Input: part model. Units: mm. Frame: model coordinates. A direction names the side the tool comes from. Round coordinates to 2 decimals unless told otherwise and drop trailing zeros. Write each loop counter-clockwise with the first axis right and the second up, starting at its lowest first coordinate (ties: lowest second). Pieces come first, ordered by that corner, then holes. Notation, with made-up numbers: (3, -21.5) -> (19, -21.5) arc R14 ccw to (19, -6.5) -> close; hole circle Ø7 at (28, -38). An arc over 180 degrees is marked (long way). Write item = value, one per line.
```python
from build123d import *

# Parameters (mm, degrees)
SKETCH_1_W      = 35
SKETCH_1_H      = 100
EXTRUDE_1_DEPTH = 10
SKETCH_2_R      = 12.5
EXTRUDE_2_DEPTH = 30
SKETCH_3_R      = 7.5
EXTRUDE_3_DEPTH = 25


with BuildPart() as part:
    # 草图1 → 凸台-拉伸1 (new body)
    with BuildSketch(Plane.XY):
        Rectangle(SKETCH_1_W, SKETCH_1_H)
    extrude(amount=EXTRUDE_1_DEPTH)

    # 草图2 → 凸台-拉伸2 (add)
    with BuildSketch(Plane.XY.offset(10)):
        with Locations(Location((0, 30, 0), (0, 0, 180))):
            Circle(SKETCH_2_R)
    extrude(amount=EXTRUDE_2_DEPTH)

    # 草图3 → 凸台-拉伸3 (add)
    with BuildSketch(Plane(origin=(0, 0, 0), x_dir=(-1, 0, 0), z_dir=(0, 0, -1))):
        with Locations((0, 30)):
            Circle(SKETCH_3_R)
    extrude(amount=EXTRUDE_3_DEPTH)


solid = part.part
```
1) Line query: L1, parallel to Z at x = 15.5, y = 22.5; L2, parallel to Z at x = 10, y = 35.5; L3, parallel to X at y = 23, z = 28. Output: solid intervals per line, ascending. Write a range as from..to.
Solutions:
L1 = 0..10
L2 = 0..40
L3 = -10.36..10.36
2) Cut plane B-B (y = 30). Return the cut outline in (x, z).
Solutions:
outline = (-17.5, 0) -> (-7.5, 0) -> (-7.5, -25) -> (7.5, -25) -> (7.5, 0) -> (17.5, 0) -> (17.5, 10) -> (12.5, 10) -> (12.5, 40) -> (-12.5, 40) -> (-12.5, 10) -> (-17.5, 10) -> close
3) Cut plane A-A (x = 0). Return the cut outline in (y, z), and give its area (4 significant figures).
Solutions:
outline = (-50, 0) -> (22.5, 0) -> (22.5, -25) -> (37.5, -25) -> (37.5, 0) -> (50, 0) -> (50, 10) -> (42.5, 10) -> (42.5, 40) -> (17.5, 40) -> (17.5, 10) -> (-50, 10) -> close
area = 2,125 mm^2
4) Cut plane C-C (z = 17). Return the cut outline in (x, y), and give its area (3 significant figures).
Solutions:
outline = circle Ø25 at (0, 30)
area = 491 mm^2
5) Access query for faces 1 (the face through (0, 30, -25)), 2 (the face through (1.63, 22.68, -12.32)), 3 (the face through (2.71, 42.203, 24.79)). Directions: +Z, -Z, +X, -X, +Y, -Y. A direction counts if a zero-diameter tool reaches every point of the face in a straight line with its end or side. Return the directions, or none.
Solutions:
face_1 = -Z, +X, -X, +Y, -Y
face_2 = -Z
face_3 = +Z
6) First-contact query: P1, Ø1.5, axis at x = -9.5, z = 18, coming from the +Y side; P2, Ø4, axis at x = 12.5, y = -28.5, coming from the +Z side; P3, Ø3, axis at x = 1.5, z = 30.5, coming from the +Y side. Flat tips, straight axial feed; report the tip coordinate or a pass-through.
Solutions:
P1 = 38.93
P2 = 10
P3 = 42.5
7) Cut plane D-D (y = -3). Return the cut outline in (x, z), and give its area (3 significant figures).
Solutions:
outline = (-17.5, 0) -> (17.5, 0) -> (17.5, 10) -> (-17.5, 10) -> close
area = 350 mm^2
